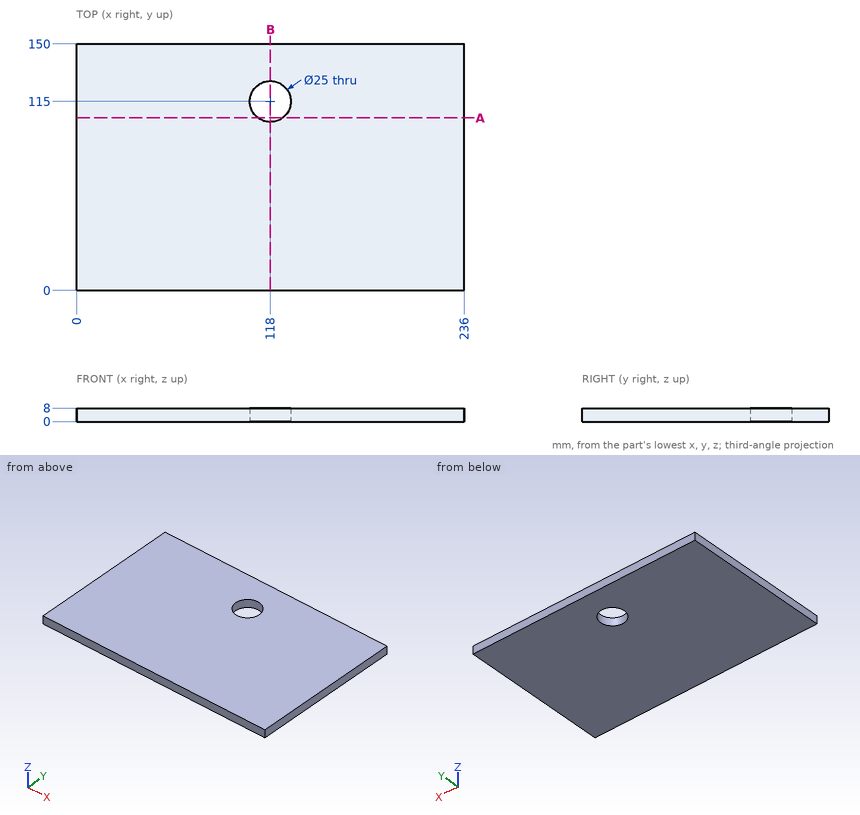
The drawing under review shows one solid part. Ordinate dimensions are in mm from its lowest x, y, z. Round coordinates to 2 decimals unless told otherwise and drop trailing zeros. Loops run counter-clockwise (first coordinate to the right, second up) from the corner with the lowest first, then second, coordinate; pieces in that order, holes last. Notation, with made-up numbers: (33.5, 13.5) -> (59.5, 13.5) arc R16 ccw to (59.5, 44.5) -> close; hole circle Ø8 at (44, -10.75). An arc over 180 degrees is marked (long way). Answer in a Markdown table with one row per item.
1) Consider section B-B, the plane x = 118. Write out the cut boundary in (y, z).
Taken from the geometry:
| item | result |
|---|---|
| outline | (0, 0) -> (102.5, 0) -> (102.5, 8) -> (0, 8) -> close; (127.5, 0) -> (150, 0) -> (150, 8) -> (127.5, 8) -> close |
2) Wall thickness on line 1 along Y through (x, z) = (118, 6.5); line 2 along Y through (x, z) = (124, 4.25): over which ranges is each line inside the solid? List them lowest first.
Taken from the geometry:
| item | result |
|---|---|
| line 1 | y = 0 to 102.5, 127.5 to 150 |
| line 2 | y = 0 to 104.03, 125.97 to 150 |
3) Consider section A-A, the plane y = 105. Write out the cut boundary in (x, z), plus the area to 3 significant figures.
Taken from the geometry:
| item | result |
|---|---|
| outline | (0, 0) -> (110.5, 0) -> (110.5, 8) -> (0, 8) -> close; (125.5, 0) -> (236, 0) -> (236, 8) -> (125.5, 8) -> close |
| area | 1,770 mm² |
